For this review, use the dimensioned drawing (mm, ordinates from the lowest corner) and the shaded views. Give positions to 0.01 mm unless a question says otherwise; leave off trailing zeros. Write each loop counter-clockwise with the first axis right and the second up, starting at its lowest first coordinate (ties: lowest second). Pieces come first, ordered by that corner, then holes.
1) For P1, Ø1, axis at x = 219.5, y = 33, coming from the -Z side; P2, Ø1.5, axis at x = 689, y = 51.5, coming from the -Z side, all flat-tipped, find the tip position at first contact; note any pin that passes through.
2) Wall thickness on line 1 along Y through (x, z) = (198, 357); line 2 along Z through (x, y) = (38.5, 57.5); line 3 along Z through (x, y) = (591, 46) (1 decimal): over which ranges is each line inside the solid? List them lowest first.
3) We need section C-C on z = 360. Give the boundary of the cut face in (x, y), and give its area (3 significant figures).
4) We need section A-A on x = 570. Give the boundary of the cut face in (y, z).
5) We need section B-B on y = 10. Give the boundary of the cut face in (x, z).
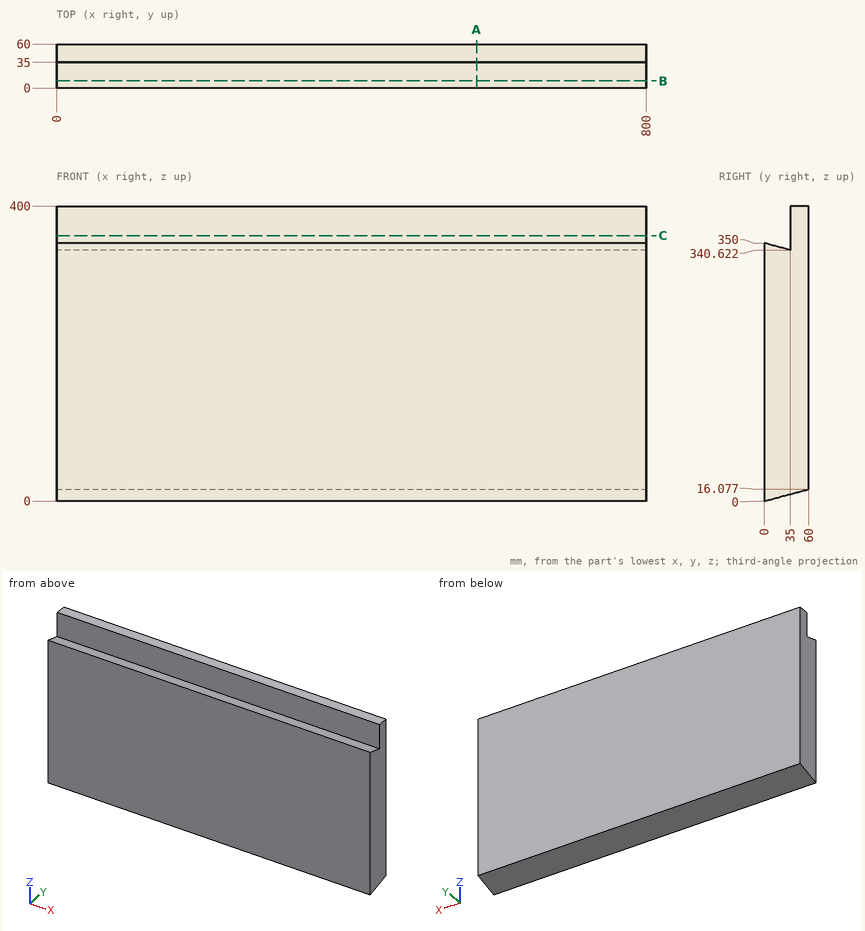
Results list:
1. P1: stops at z = 8.71
1. P2: stops at z = 13.6
2. line 1: y = 35 to 60
2. line 2: z = 15.41 to 400
2. line 3: z = 12.3 to 400
3. outline: (0, 35) - (800, 35) - (800, 60) - (0, 60) - close
3. area: 20,000 mm2
4. outline: (0, 0) - (60, 16.08) - (60, 400) - (35, 400) - (35, 340.62) - (0, 350) - close
5. outline: (0, 2.68) - (800, 2.68) - (800, 347.32) - (0, 347.32) - close
